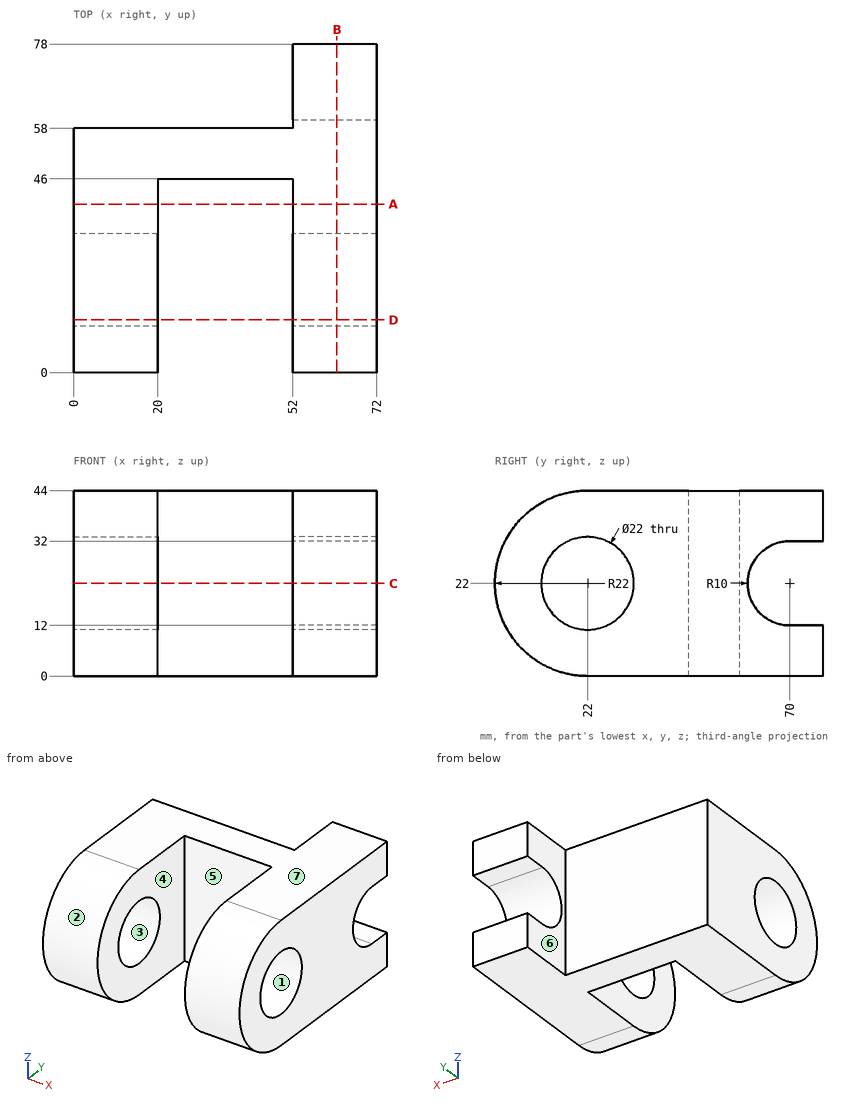
Could you check a few things on this drawing? It's one solid part, dimensions in mm from its lowest x, y, z. A direction names the side the tool comes from. Give positions to 0.01 mm unless a question says otherwise; leave off trailing zeros. Order: outer loops, then holes, each group sorted by start corner. A loop starts at its lowest first (then second) coordinate and runs counter-clockwise, first axis right, second up. Notation, with made-up numbers: (10, -4.5) -> (20, -4.5) arc R22 ccw to (20, 25.5) -> close; hole circle Ø10 at (45, 37). An arc over 180 degrees is marked (long way). Answer in a Markdown table with one row per item. Add a question column.
Item 1: Imagine slicing it at B-B (x = 62.5). List the corners of the cut face in (y, z) for me, and give its area (3 significant figures).
Item 2: For the marked faces 5, 6 and 7, which set-ups out of +Z, -Z, +X, -X, +Y, -Y let a thin tool reach every point of the face, with its end or its side?
Item 3: Imagine slicing it at A-A (y = 40). List the corners of the cut face in (x, z) for me.
Item 4: Imagine slicing it at C-C (z = 22). List the corners of the cut face in (x, y) for me.
Item 5: Imagine slicing it at D-D (y = 12.5). List the corners of the cut face in (x, z) for me, and give its area (3 significant figures).
Item 6: We'd pull the mould along Y, two halves only. Please class the marked faces 1, 2, 3 and 4: pulls with the +Y half, pulls with the -Y half, needs draft (parallel to the pull), parting line crosses it, or undercut.
Item 7: I'm going to push a flat-ended pin straight in: P1, Ø2, axis at x = 58.5, y = 13.5, coming from the -Z side. Where does the tip first touch, or does it pass through?
Item 8: Please list where these lines run through material, in increasing order: probe 1 along Y at (x, z) = (58, 22); probe 2 along X at (y, z) = (37.5, 23); probe 3 along Y at (x, z) = (6.75, 22).
Result:
| question | item | result |
|---|---|---|
| 1 | outline | (22, 0) -> (78, 0) -> (78, 12) -> (70, 12) arc R10 cw to (70, 32) -> (78, 32) -> (78, 44) -> (22, 44) arc R22 ccw to start; hole circle Ø22 at (22, 22) |
| 1 | area | 2,530 mm2 |
| 2 | face 5 | +Z, -Z, -Y |
| 2 | face 6 | +Z, -Z, -X, +Y |
| 2 | face 7 | +Z, +X, -X, +Y, -Y |
| 3 | outline | (0, 0) -> (20, 0) -> (20, 44) -> (0, 44) -> close; (52, 0) -> (72, 0) -> (72, 44) -> (52, 44) -> close |
| 4 | outline | (0, 0) -> (20, 0) -> (20, 11) -> (0, 11) -> close; (0, 33) -> (20, 33) -> (20, 46) -> (52, 46) -> (52, 33) -> (72, 33) -> (72, 60) -> (52, 60) -> (52, 58) -> (0, 58) -> close; (52, 0) -> (72, 0) -> (72, 11) -> (52, 11) -> close |
| 5 | outline | (0, 2.16) -> (20, 2.16) -> (20, 16.45) -> (0, 16.45) -> close; (0, 27.55) -> (20, 27.55) -> (20, 41.84) -> (0, 41.84) -> close; (52, 2.16) -> (72, 2.16) -> (72, 16.45) -> (52, 16.45) -> close; (52, 27.55) -> (72, 27.55) -> (72, 41.84) -> (52, 41.84) -> close |
| 5 | area | 1,140 mm2 |
| 6 | face 1 | undercut |
| 6 | face 2 | pulls with the -Y half |
| 6 | face 3 | undercut |
| 6 | face 4 | needs draft |
| 7 | P1 | z = 1.32 |
| 8 | probe 1 | 0 to 11, 33 to 60 |
| 8 | probe 2 | 0 to 20, 52 to 72 |
| 8 | probe 3 | 0 to 11, 33 to 58 |
